Verification items for the finished model (mm, model axes). Round coordinates to 2 decimals unless told otherwise and drop trailing zeros. Order: outer loops, then holes, each group sorted by start corner. A loop starts at its lowest first (then second) coordinate and runs counter-clockwise, first axis right, second up.
```python
from build123d import *

# Parameters (mm, degrees)
SKETCH1_W                    = 190
SKETCH1_H                    = 30
BOSS_EXTRUDE1_DEPTH          = 10
CHAMFER1_SIZE                = 3
F_9_0_9_DIAMETER_HOLE1_D     = 9
F_9_0_9_DIAMETER_HOLE1_DEPTH = 19.75
F_9_0_9_DIAMETER_HOLE1_TIP   = 2.703872786
F_9_0_9_DIAMETER_HOLE2_D     = 12
F_9_0_9_DIAMETER_HOLE2_DEPTH = 19.75
F_9_0_9_DIAMETER_HOLE2_TIP   = 3.605163714


with BuildPart() as part:
    # Sketch1 → Boss-Extrude1 (new body)
    with BuildSketch(Plane(origin=(0, 0, 0), x_dir=(1, 0, 0), z_dir=(0, 1, 0))):
        Rectangle(SKETCH1_W, SKETCH1_H)
    extrude(amount=BOSS_EXTRUDE1_DEPTH)

    # Chamfer1
    chamfer1_edges = [part.edges().sort_by_distance(p)[0] for p in [
        (95, 5, 15),
        (-95, 5, 15),
        (-95, 5, -15),
        (95, 5, -15),
    ]]
    chamfer(chamfer1_edges, length=CHAMFER1_SIZE)

    # Ø9.0 (9) Diameter Hole1
    with Locations(Plane(origin=(0, 10, 0), x_dir=(1, 0, 0), z_dir=(0, 1, 0))):
        with Locations((85, 0), (70, 0), (55, 0)):
            Hole(F_9_0_9_DIAMETER_HOLE1_D / 2, depth=F_9_0_9_DIAMETER_HOLE1_DEPTH)
            with Locations((0, 0, -(F_9_0_9_DIAMETER_HOLE1_DEPTH + F_9_0_9_DIAMETER_HOLE1_TIP / 2))):  # 118° drill point
                Cone(0, F_9_0_9_DIAMETER_HOLE1_D / 2, F_9_0_9_DIAMETER_HOLE1_TIP, mode=Mode.SUBTRACT)

    # Ø9.0 (9) Diameter Hole2
    with Locations(Plane(origin=(0, 0, 0), x_dir=(-1, 0, 0), z_dir=(0, -1, 0))):
        with Locations((78.492424049, 0)):
            Hole(F_9_0_9_DIAMETER_HOLE2_D / 2, depth=F_9_0_9_DIAMETER_HOLE2_DEPTH)
            with Locations((0, 0, -(F_9_0_9_DIAMETER_HOLE2_DEPTH + F_9_0_9_DIAMETER_HOLE2_TIP / 2))):  # 118° drill point
                Cone(0, F_9_0_9_DIAMETER_HOLE2_D / 2, F_9_0_9_DIAMETER_HOLE2_TIP, mode=Mode.SUBTRACT)


solid = part.part
```
1) Sectioned sample at A-A on x = 85. Record the cut outline in (y, z), then the cut area to 3 significant figures.
2) Sectioned sample at B-B on y = 3.25. Record the cut outline in (x, z), then the cut area to 3 significant figures.
3) Scan lines: probe 1 along Z at (x, y) = (55, 4.5); probe 2 along Z at (x, y) = (-78, 5.75); probe 3 along X at (y, z) = (4, 1). Record each from-to range of solid material in increasing order.
4) Draft check along X on faces 1 (the cylindrical face through (65.84, 4.93, 1.72)), 2 (the flat face through (-1, 0, 0)), 3 (the flat face through (-95, 5, 0)). Enter one of: released by +X, released by -X, zero draft, split by the parting line, or undercut.
Returned:
1. outline: (0, -15) - (10, -15) - (10, -4.5) - (0, -4.5) - close; (0, 4.5) - (10, 4.5) - (10, 15) - (0, 15) - close
1. area: 210 mm2
2. outline: (-95, -12) - (-92, -15) - (92, -15) - (95, -12) - (95, 12) - (92, 15) - (-92, 15) - (-95, 12) - close; hole circle Ø12 at (-78.49, 0); hole circle Ø9 at (55, 0); hole circle Ø9 at (70, 0); hole circle Ø9 at (85, 0)
2. area: 5,380 mm2
3. probe 1: z = -15 to -4.5, 4.5 to 15
3. probe 2: z = -15 to -5.98, 5.98 to 15
3. probe 3: x = -95 to -84.41, -72.58 to 50.61, 59.39 to 65.61, 74.39 to 80.61, 89.39 to 95
4. face 1: undercut
4. face 2: zero draft
4. face 3: released by -X
